Read the model definition and answer for the solid it produces. Units are mm, in the model's axes. A direction names the side the tool comes from. Coordinates: 2 decimals unless noted, no trailing zeros. Write each loop counter-clockwise with the first axis right and the second up, starting at its lowest first coordinate (ties: lowest second). Pieces come first, ordered by that corner, then holes. Notation, with made-up numbers: (49.25, 28) -> (92.25, 28) arc R35 ccw to (92.25, 60) -> close; hole circle Ø11 at (-6, 30). An arc over 180 degrees is marked (long way). Answer as a JSON object with one key per item and string values. Group by question number.
(1) Straight lines are drawn through the part: L1, parallel to X at y = 38.5, z = 0; L2, parallel to X at y = 26, z = 0; L3, parallel to Y at x = -60, z = 30.5. For each, find the intervals that lie inside material, in ascending order.
(2) Find section C-C (x = 98.5). Give the vertices of the cut face in (y, z).
(3) Find section B-B (z = -16). Give the vertices of the cut face in (x, y).
(4) For a pull along Y with two mould halves and no side action, classify faces 1 (the face through (-36, 30, 35)), 2 (the face through (60, 10, -18)), 3 (the face through (-57, 45, 28)) as +Y half, -Y half, draft (parallel to the pull), parting line (faces both ways), or undercut.
(5) Flat-ended cylindrical pins translate along their axes: P1, Ø12, axis at x = 42, y = 18.5, coming from the +Z side; P2, Ø10, axis at x = 75, z = 15.5, coming from the +Y side; P3, Ø5, axis at x = 20, y = 48, coming from the +Z side. Find the tip coordinate at first contact, or state that the pin passes through.
(6) Which of the six approach directions +Z, -Z, +X, -X, +Y, -Y give full straight-line access (tool end or side, diameter ignored) to faces 4 (the face through (32.62, 29.58, 12.69)), 5 (the face through (70.44, 4.93, -29.62)), 6 (the face through (-34, 30, -35))?
(7) Find section D-D (y = 12.5). Give the vertices of the cut face in (x, z).
(8) Find section A-A (y = 27). Give the vertices of the cut face in (x, z).
from build123d import *

# Parameters (mm, degrees)
BASE_BLOCK_DEPTH              = 60
BLOCK_SIDE_PROFILE_CUT_DEPTH  = 129.840987267
VERTICAL_BORE_SKETCH_R        = 20
VERTICAL_BORE_40_DEPTH        = 114.688170009
HORIZONTAL_BORE_SKETCH_R      = 15
HORIZONTAL_BORE_30_DEPTH      = 129.840987267
COUNTERBORE_SIDE_A_SKETCH_R   = 20
COUNTERBORE_SIDE_A_40X7_DEPTH = 7
COUNTERBORE_START             = -7
COUNTERBORE_SIDE_B_SKETCH_R   = 20
COUNTERBORE_SIDE_B_40X7_DEPTH = 7
FORK_ARM_DEPTH                = 20
ARM_WEB_PLATE_DEPTH           = 10
ARM_RIB_REACH                 = 142
ARM_RIB_SKETCH_WALL_W         = 333.478150704
ARM_RIB_SKETCH_WALL_H         = 10


with BuildPart() as part:
    # Base Block Sketch → Base Block (new body)
    with BuildSketch(Plane(origin=(0, 0, 0), x_dir=(1, 0, 0), z_dir=(0, 1, 0))):
        with BuildLine():
            Line((0, 35), (-90, 35))
            Line((-90, 35), (-90, -35))
            Line((-90, -35), (0, -35))
            ThreePointArc((0, -35), (35, 0), (0, 35))
        make_face()
    extrude(amount=BASE_BLOCK_DEPTH)

    # Block Side Profile Sketch → Block Side Profile Cut (cut, through all)
    with BuildSketch(Plane.XY.offset(35)):
        with BuildLine():
            Line((-60, 60), (-120, 60))
            Line((-120, 60), (-120, 0))
            Line((-120, 0), (-60, 0))
            ThreePointArc((-60, 0), (-90, 30), (-60, 60))
        make_face()
    extrude(amount=-BLOCK_SIDE_PROFILE_CUT_DEPTH, mode=Mode.SUBTRACT)

    # Vertical Bore Sketch → Vertical Bore Ø40 (cut, through all)
    with BuildSketch(Plane(origin=(0, 60, 0), x_dir=(1, 0, 0), z_dir=(0, 1, 0))):
        with Locations(Location((0, 0, 0), (0, 0, 270))):
            Circle(VERTICAL_BORE_SKETCH_R)
    extrude(amount=-VERTICAL_BORE_40_DEPTH, mode=Mode.SUBTRACT)

    # Horizontal Bore Sketch → Horizontal Bore Ø30 (cut, through all)
    with BuildSketch(Plane.XY.offset(35)):
        with Locations((-60, 30)):
            Circle(HORIZONTAL_BORE_SKETCH_R)
    extrude(amount=-HORIZONTAL_BORE_30_DEPTH, mode=Mode.SUBTRACT)

    # Counterbore Side A Sketch → Counterbore Side A Ø40x7 (cut)
    with BuildSketch(Plane.XY.offset(35)):
        with Locations((-60, 30)):
            Circle(COUNTERBORE_SIDE_A_SKETCH_R)
    extrude(amount=-COUNTERBORE_SIDE_A_40X7_DEPTH, mode=Mode.SUBTRACT)

    # Counterbore Side B Sketch → Counterbore Side B Ø40x7 (cut)
    with BuildSketch(Plane(origin=(0, 0, -35), x_dir=(-1, 0, 0), z_dir=(0, 0, -1)).offset(COUNTERBORE_START)):
        with Locations(Location((60, 30, 0), (0, 0, 180))):
            Circle(COUNTERBORE_SIDE_B_SKETCH_R)
    extrude(amount=COUNTERBORE_SIDE_B_40X7_DEPTH, mode=Mode.SUBTRACT)



with BuildPart() as body_2:
    # Fork Arm Sketch → Fork Arm (new body)
    with BuildSketch(Plane(origin=(0, 0, 0), x_dir=(1, 0, 0), z_dir=(0, 1, 0))):
        with BuildLine():
            Line((120, 40), (120, 25))
            ThreePointArc((120, 25), (95, 0), (120, -25))
            Line((120, -25), (120, -40))
            ThreePointArc((120, -40), (80, 0), (120, 40))
        make_face()
    extrude(amount=FORK_ARM_DEPTH)


with BuildPart() as part_1:
    add(part.part)

    add(body_2.part)  # Arm Web Plate merges body 2
    # Arm Web Plate Sketch → Arm Web Plate (add)
    with BuildSketch(Plane(origin=(0, 0, 0), x_dir=(1, 0, 0), z_dir=(0, 1, 0))):
        with BuildLine():
            Line((111.011327845, 38.976964644), (28.722813233, 20))
            ThreePointArc((28.722813233, 20), (35, 0), (28.722813233, -20))
            Line((28.722813233, -20), (111.011327845, -38.976964644))
            ThreePointArc((111.011327845, -38.976964644), (80, 0), (111.011327845, 38.976964644))
        make_face()
    extrude(amount=ARM_WEB_PLATE_DEPTH)

    # Arm Rib Sketch wall → Arm Rib (add, up to next)
    with BuildSketch(Plane(origin=(57.5, 32.5, 0), x_dir=(0.874157276122, -0.485642931179, 0), z_dir=(0.485642931179, 0.874157276122, 0)), mode=Mode.PRIVATE) as arm_rib_sk1:
        Rectangle(ARM_RIB_SKETCH_WALL_W, ARM_RIB_SKETCH_WALL_H)
    arm_rib_tool1 = extrude(arm_rib_sk1.sketch, amount=-ARM_RIB_REACH, mode=Mode.PRIVATE) - part_1.part
    add(arm_rib_tool1.solids().sort_by_distance((57.5, 32.5, 0))[0])


solid = part_1.part
Results below:
{
 "1": {"L1": "x = -88.77 to -72.36, -47.64 to -20, 20 to 46.7", "L2": "x = -89.73 to -74.46, -45.54 to -20, 20 to 69.2", "L3": "y = 0 to 10, 50 to 60"},
 "2": {"outline": "(0, -36.09) -> (10, -36.09) -> (10, -33.73) -> (20, -33.73) -> (20, -12.76) -> (0, -12.76) -> close; (0, 12.76) -> (20, 12.76) -> (20, 33.73) -> (10, 33.73) -> (10, 36.09) -> (0, 36.09) -> close"},
 "3": {"outline": "(-60, 0) -> (-12, 0) -> (-12, 60) -> (-60, 60) arc R30 ccw to start; (12, 0) -> (100.79, 0) -> (100.79, 20) -> (83.34, 20) -> (83.34, 10) -> (31.13, 10) -> (31.13, 60) -> (12, 60) -> close; hole circle Ø30 at (-60, 30)"},
 "4": {"face 1": "draft", "face 2": "+Y half", "face 3": "undercut"},
 "5": {"P1": "stops at z = 5", "P2": "stops at y = 10", "P3": "stops at z = 30.31"},
 "6": {"face 4": "+Y", "face 5": "-Z, +Y, -Y", "face 6": "-Z, -X, +Y, -Y"},
 "7": {"outline": "(-84.37, -35) -> (-69.68, -35) -> (-69.68, -28) -> (-50.32, -28) -> (-50.32, -35) -> (0, -35) arc R35 ccw to (34.64, -5) -> (80.31, -5) arc R40 ccw to (120, -40) -> (120, -25) arc R25 cw to (120, 25) -> (120, 40) arc R40 ccw to (80.31, 5) -> (34.64, 5) arc R35 ccw to (0, 35) -> (-50.32, 35) -> (-50.32, 28) -> (-69.68, 28) -> (-69.68, 35) -> (-84.37, 35) -> close; hole circle Ø40 at (0, 0)"},
 "8": {"outline": "(-89.85, -35) -> (-79.77, -35) -> (-79.77, -28) -> (-74.7, -28) -> (-74.7, 28) -> (-79.77, 28) -> (-79.77, 35) -> (-89.85, 35) -> close; (-45.3, -28) -> (-40.23, -28) -> (-40.23, -35) -> (0, -35) arc R35 ccw to (34.64, -5) -> (67.4, -5) -> (67.4, 5) -> (34.64, 5) arc R35 ccw to (0, 35) -> (-40.23, 35) -> (-40.23, 28) -> (-45.3, 28) -> close; hole circle Ø40 at (0, 0)"}
}
